Part model, mm, in its own coordinate system. Face numbers are marked on the shaded views. A direction names the side the tool comes from. Give positions to 0.01 mm unless a question says otherwise; leave off trailing zeros. Write each loop counter-clockwise with the first axis right and the second up, starting at its lowest first coordinate (ties: lowest second). Pieces come first, ordered by that corner, then holes.
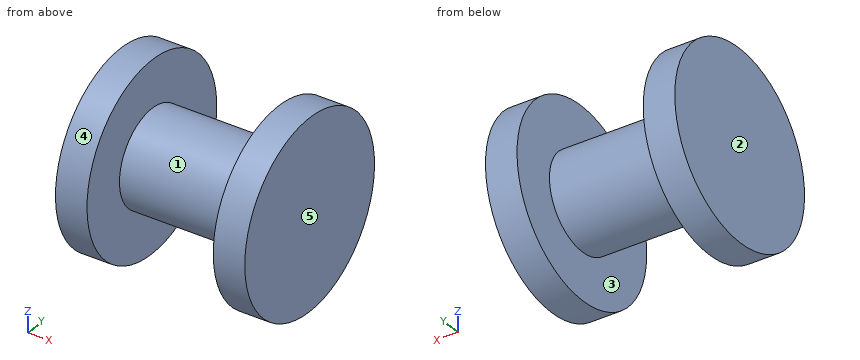
from build123d import *

# Parameters (mm, degrees)
SCALE1_SCALE = 0.3


with BuildPart() as part:
    # Sketch2 → Revolve1 (revolve)
    with BuildSketch(Plane.XY, mode=Mode.PRIVATE) as revolve1_sk:
        Polygon((10, -7.5), (10, -15), (15, -15), (15, 0), (-15, 0), (-15, -15), (-10, -15), (-10, -7.5), align=None)
    revolve(revolve1_sk.sketch.rotate(Axis((15, 0, 0), (-1, 0, 0)), 270), axis=Axis((15, 0, 0), (-1, 0, 0)))


with BuildPart() as part_1:
    # Scale1: scaled about (0, 0, 0)
    add(part.part.scale(SCALE1_SCALE))


solid = part_1.part
1) Flat gauge pins, fed straight in: P1, Ø1, axis at x = -3, y = 1.5, coming from the -Z side; P2, Ø1.5, axis at x = -0.5, z = 1, coming from the +Y side; P3, Ø2, axis at x = 2.5, z = -1, coming from the +Y side. Where does each tip first touch, or does it go through?
Check result:
P1: stops at z = -4.39
P2: stops at y = 2.24
P3: stops at y = 4.5
2) Saw through at D-D (y = -3.25). Write the cut outline in (x, z).
Check result:
outline: (-4.5, -3.11) - (-3, -3.11) - (-3, 3.11) - (-4.5, 3.11) - close; (3, -3.11) - (4.5, -3.11) - (4.5, 3.11) - (3, 3.11) - close
3) Saw through at B-B (z = 2.5). Write the cut outline in (x, y), and give its area (4 significant figures).
Check result:
outline: (-4.5, -3.74) - (-3, -3.74) - (-3, 3.74) - (-4.5, 3.74) - close; (3, -3.74) - (4.5, -3.74) - (4.5, 3.74) - (3, 3.74) - close
area: 22.45 mm2
4) Mould opens along X. For the marked faces 3, 4 and 5 say: +X half, -X half, draft (parallel to the pull), parting line (faces both ways), or undercut.
Check result:
face 3: undercut
face 4: draft
face 5: +X half
5) Drill centre lines: L1, parallel to X at y = 0.25, z = 3; L2, parallel to Y at x = -3.5, z = -1.5; L3, parallel to Z at x = -2.25, y = 2. Where is each one in solid material? Low to high.
Check result:
L1: x = -4.5 to -3, 3 to 4.5
L2: y = -4.24 to 4.24
L3: z = -1.03 to 1.03
6) Saw through at A-A (y = 0). Write the cut outline in (x, z).
Check result:
outline: (-4.5, -4.5) - (-3, -4.5) - (-3, -2.25) - (3, -2.25) - (3, -4.5) - (4.5, -4.5) - (4.5, 4.5) - (3, 4.5) - (3, 2.25) - (-3, 2.25) - (-3, 4.5) - (-4.5, 4.5) - close
7) 3-axis set-ups, long thin cutter, end or side, ignore diameter. For the marked faces 1 and 2: which of +Z, -Z, +X, -X, +Y, -Y reach the whole face in a straight line?
Check result:
face 1: none
face 2: +Z, -Z, -X, +Y, -Y
